Can you work these out from the model? Positions are in its coordinate system, mm. Coordinates: 2 decimals unless noted, no trailing zeros. Write each loop counter-clockwise with the first axis right and the second up, starting at its lowest first coordinate (ties: lowest second). Pieces come first, ordered by that corner, then holes. Notation, with made-up numbers: (46.5, 81) -> (56.5, 81) arc R37 cw to (56.5, 119) -> close; hole circle Ø11 at (48.25, -17). An arc over 180 degrees is marked (long way). Answer as CSV lines item,"result". Start each with the question number.
```python
from build123d import *

# Parameters (mm, degrees)
EXTRUDE_1_DEPTH     = 8
SKETCH_5_R          = 10
CUT_EXTRUDE_1_DEPTH = 25.269322199


with BuildPart() as part:
    # 草图1 → 凸台-拉伸1 (new body)
    with BuildSketch(Plane.XY):
        Polygon((0, 17.320508076), (-15, 8.660254038), (-15, -8.660254038), (0, -17.320508076), (15, -8.660254038), (15, 8.660254038), align=None)
    extrude(amount=EXTRUDE_1_DEPTH)

    # 草图4 → 切除-旋转1 (revolve, cut)
    with BuildSketch(Plane(origin=(0, 0, 0), x_dir=(0, 0, -1), z_dir=(1, 0, 0)), mode=Mode.PRIVATE) as cut_revolve_1_sk:
        Polygon((-8, -13.5), (-6.609448781, -17.320508076), (-8, -17.320508076), align=None)
    cut_revolve_1 = revolve(cut_revolve_1_sk.sketch.rotate(Axis((0, 0, 8), (0, 0, -1)), 120.000000002), axis=Axis((0, 0, 8), (0, 0, -1)), mode=Mode.SUBTRACT)

    # 镜向1: 切除-旋转1 across plane
    add(cut_revolve_1.mirror(Plane.XY.offset(4)), mode=Mode.SUBTRACT)

    # 草图5 → 切除-拉伸1 (cut, through all)
    with BuildSketch(Plane.XY.offset(8)):
        Circle(SKETCH_5_R)
    extrude(amount=-CUT_EXTRUDE_1_DEPTH, mode=Mode.SUBTRACT)


solid = part.part
```
Q1. I need wall thicknesses on L1, parallel to X at y = 5, z = 2.75; L2, parallel to Y at x = 3, z = 5.5; L3, parallel to X at y = -6, z = 4.5. Which ranges of each line are inside material? Lowest first, please.
Q2. Imagine slicing it at C-C (z = 1). Write out the boundary of the cut face in (x, y), then the cut area to 3 significant figures.
Q3. Imagine slicing it at B-B (y = 0). Write out the boundary of the cut face in (x, z), then the cut area to 3 significant figures.
Q4. If we mould it in two halves opening along Y, with no side actions, what happens to faces 1 (the face through (7.605, 12.93, 3.952)), 2 (the face through (-2.17, -9.76, 4.06)), 3 (the face through (15, 0, 4))? For each: released by +Y, released by -Y, zero draft, split by the parting line, or undercut.
Q5. Imagine slicing it at A-A (z = 4.5). Write out the boundary of the cut face in (x, y).
Q6. For pin 1 (3 mm diameter, centred on x = -4, z = 3, fed in from +Y); pin 2 (1.5 mm diameter, centred on x = 9.5, z = 3.5, fed in from +Y); pin 3 (2 mm diameter, centred on x = -4.5, z = 4, fed in from +Y), each with a flat end and sliding along its axis, tell me the tip position at first contact or that it passes through.
Entries:
1,L1,"-15 to -8.66, 8.66 to 15"
1,L2,"-15.59 to -9.54, 9.54 to 15.59"
1,L3,"-15 to -8, 8 to 15"
2,outline,"(-15, -6.24) arc R16.25 ccw to (-12.91, -9.87) -> (-2.09, -16.11) arc R16.25 ccw to (2.09, -16.11) -> (12.91, -9.87) arc R16.25 ccw to (15, -6.24) -> (15, 6.24) arc R16.25 ccw to (12.91, 9.87) -> (2.09, 16.11) arc R16.25 ccw to (-2.09, 16.11) -> (-12.91, 9.87) arc R16.25 ccw to (-15, 6.24) -> close; hole circle Ø20 at (0, 0)"
2,area,"452 mm2"
3,outline,"(-15, 0.55) -> (-13.5, 0) -> (-10, 0) -> (-10, 8) -> (-13.5, 8) -> (-15, 7.45) -> close; (10, 0) -> (13.5, 0) -> (15, 0.55) -> (15, 7.45) -> (13.5, 8) -> (10, 8) -> close"
3,area,"78.4 mm2"
4,face 1,"released by +Y"
4,face 2,"undercut"
4,face 3,"zero draft"
5,outline,"(-15, -8.66) -> (0, -17.32) -> (15, -8.66) -> (15, 8.66) -> (0, 17.32) -> (-15, 8.66) -> close; hole circle Ø20 at (0, 0)"
6,pin 1,"y = 15.88"
6,pin 2,"y = 12.27"
6,pin 3,"y = 15.3"
